from build123d import *

# Parameters (mm, degrees)
SKETCH_1_W      = 598.5
SKETCH_1_H      = 1319
EXTRUDE_1_DEPTH = 28
SHELL_1_T       = -2
SKETCH_2_W      = 598.5
SKETCH_2_H      = 1319
SKETCH_2_W_2    = 558.5
SKETCH_2_H_2    = 1279
EXTRUDE_2_DEPTH = 2


with BuildPart() as part:
    # 草图1 → 凸台-拉伸1 (new body)
    with BuildSketch(Plane.XY):
        with Locations((299.25, 659.5)):
            Rectangle(SKETCH_1_W, SKETCH_1_H)
    extrude(amount=EXTRUDE_1_DEPTH)

    # 抽壳1
    shell_1_openings = [part.faces().sort_by_distance(p)[0] for p in [
        (299.25, 659.5, 28),
    ]]
    offset(amount=SHELL_1_T, openings=shell_1_openings, kind=Kind.INTERSECTION)

    # 草图2 → 凸台-拉伸2 (add)
    with BuildSketch(Plane.XY.offset(28)):
        with Locations((299.25, 659.5)):
            Rectangle(SKETCH_2_W, SKETCH_2_H)
        with Locations((299.25, 659.5)):
            Rectangle(SKETCH_2_W_2, SKETCH_2_H_2, mode=Mode.SUBTRACT)
    extrude(amount=-EXTRUDE_2_DEPTH)


solid = part.part
Part model, mm, in its own coordinate system. A direction names the side the tool comes from. Round coordinates to 2 decimals unless told otherwise and drop trailing zeros. Loops run counter-clockwise (first coordinate to the right, second up) from the corner with the lowest first, then second, coordinate; pieces in that order, holes last. Notation, with made-up numbers: (74, -37) - (93, -37) arc R30 cw to (93, -11) - close; hole circle Ø4 at (80, 15.5). An arc over 180 degrees is marked (long way). Answer as a JSON object with one key per item and string values.
Item 1: Band-saw the part on B-B on y = 1225. List the corners of the cut face in (x, z).
Output:
{"outline": "(0, 0) - (598.5, 0) - (598.5, 28) - (578.5, 28) - (578.5, 26) - (596.5, 26) - (596.5, 2) - (2, 2) - (2, 26) - (20, 26) - (20, 28) - (0, 28) - close"}
Item 2: Band-saw the part on C-C on x = 161. List the corners of the cut face in (y, z).
Output:
{"outline": "(0, 0) - (1319, 0) - (1319, 28) - (1299, 28) - (1299, 26) - (1317, 26) - (1317, 2) - (2, 2) - (2, 26) - (20, 26) - (20, 28) - (0, 28) - close"}
Item 3: Wall check: L1, parallel to X at y = 1168, z = 20.5; L2, parallel to Y at x = 486.5, z = 4.75; L3, parallel to Z at x = 152, y = 1128.5. Give the ranges that are in metal, low to high.
Output:
{"L1": "0 to 2, 596.5 to 598.5", "L2": "0 to 2, 1317 to 1319", "L3": "0 to 2"}
Item 4: Band-saw the part on A-A on z = 17. List the corners of the cut face in (x, y).
Output:
{"outline": "(0, 0) - (598.5, 0) - (598.5, 1319) - (0, 1319) - close; hole (2, 2) - (596.5, 2) - (596.5, 1317) - (2, 1317) - close"}
Item 5: Pull direction Y, two halves, no side cores. Call faces 1 (the face through (295, 1319, 14)), 2 (the face through (295, 669, 0)), 3 (the face through (2, 650, 14)), 4 (the face through (295, 0, 14)): pulls with the +Y half, pulls with the -Y half, needs draft (parallel to the pull), parting line crosses it, or undercut.
Output:
{"face 1": "pulls with the +Y half", "face 2": "needs draft", "face 3": "undercut", "face 4": "pulls with the -Y half"}
Item 6: Pin check, flat tip, straight feed: pin 1 (1.5 mm diameter, centred on x = 275, y = 570.5, fed in from +Z). Stop position of the tip, or through.
Output:
{"pin 1": "z = 2"}
Item 7: Tool access for faces 5 (the face through (586, 663, 28)), 6 (the face through (295, 1317, 14)): list every direction of +Z, -Z, +X, -X, +Y, -Y with a clear straight run to the whole face (end or side of a thin tool).
Output:
{"face 5": "+Z, +X, -X, +Y, -Y", "face 6": "none"}
